```python
from build123d import *

# Parameters (mm, degrees)
FILLET_1_R                           = 18
FILLET_2_R                           = 4
SKETCH_2_R                           = 13
CUT_EXTRUDE_1_DEPTH                  = 440.177071421
CHAMFER_1_SIZE                       = 2
PATTERN_CIRCULAR_1_COUNT             = 10
CHAMFER_1_OF_PATTERN_CIRCULAR_1_SIZE = 2


with BuildPart() as part:
    # 草图1 → 旋转1 (revolve)
    with BuildSketch(Plane.XY, mode=Mode.PRIVATE) as revolve_1_sk:
        Polygon((0, 309.5), (36, 309.5), (36, 140.5), (24, 140.5), (24, 217.5), (22, 217.5), (22, 295.5), (0, 295.5), align=None)
    revolve(revolve_1_sk.sketch.rotate(Axis((-295.4, 0, 0), (1, 0, 0)), 90), axis=Axis((-295.4, 0, 0), (1, 0, 0)))

    # 圆角1
    fillet_1_edges = [part.edges().sort_by_distance(p)[0] for p in [
        (36, 0, -309.5),
    ]]
    fillet(fillet_1_edges, radius=FILLET_1_R)

    # 圆角2
    fillet_2_edges = [part.edges().sort_by_distance(p)[0] for p in [
        (22, 0, -295.5),
    ]]
    fillet(fillet_2_edges, radius=FILLET_2_R)

    # 草图2 → 切除-拉伸1 (cut, through all)
    with BuildSketch(Plane(origin=(36, 0, 0), x_dir=(0, 0, -1), z_dir=(1, 0, 0))):
        with Locations((0, 167.5)):
            Circle(SKETCH_2_R)
    cut_extrude_1 = extrude(amount=-CUT_EXTRUDE_1_DEPTH, mode=Mode.SUBTRACT)

    # 倒角1
    chamfer_1_edges = [part.edges().sort_by_distance(p)[0] for p in [
        (24, 167.5, 13),
    ]]
    chamfer(chamfer_1_edges, length=CHAMFER_1_SIZE)

    # 草图3 → 切除-旋转1 (revolve, cut)
    with BuildSketch(Plane.XY, mode=Mode.PRIVATE) as cut_revolve_1_sk:
        with BuildLine():
            Line((32.398120874, 180.50807098), (32.398120874, 167.5))
            Line((32.398120874, 167.5), (65.246950766, 167.5))
            ThreePointArc((65.246950766, 167.5), (53.242386137, 185.165329999), (32.398120874, 180.50807098))
        make_face()
    cut_revolve_1 = revolve(cut_revolve_1_sk.sketch.rotate(Axis((0, 167.5, 0), (1, 0, 0)), 270), axis=Axis((0, 167.5, 0), (1, 0, 0)), mode=Mode.SUBTRACT)

    # 阵列(圆周)1: 切除-拉伸1, 切除-旋转1 ×10 about axis
    pattern_circular_1_axis = Axis((0, 0, 0), (1, 0, 0))
    add([cut_extrude_1.rotate(pattern_circular_1_axis, i * 360 / PATTERN_CIRCULAR_1_COUNT) for i in range(1, PATTERN_CIRCULAR_1_COUNT)], mode=Mode.SUBTRACT)
    add([cut_revolve_1.rotate(pattern_circular_1_axis, i * 360 / PATTERN_CIRCULAR_1_COUNT) for i in range(1, PATTERN_CIRCULAR_1_COUNT)], mode=Mode.SUBTRACT)

    # 倒角1 of 阵列(圆周)1
    chamfer_1_of_pattern_circular_1_edges = [part.edges().sort_by_distance(p)[0] for p in [
        (24, 127.869138278, 108.971250686),
        (24, 39.396611846, 163.319187406),
        (24, -64.12408127, 155.284745553),
        (24, -143.151554838, 87.936808832),
        (24, -167.5, -13),
        (24, -127.869138278, -108.971250686),
        (24, -39.396611846, -163.319187406),
        (24, 64.12408127, -155.284745553),
        (24, 143.151554838, -87.936808832),
    ]]
    chamfer(chamfer_1_of_pattern_circular_1_edges, length=CHAMFER_1_OF_PATTERN_CIRCULAR_1_SIZE)


solid = part.part
```
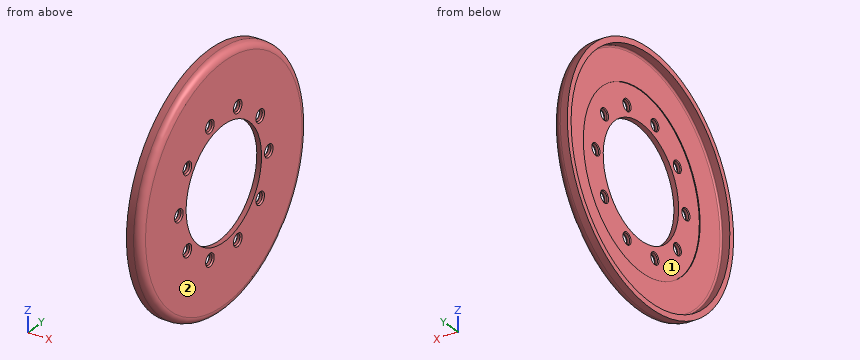
Work out the finished part from the listing and answer in its coordinate system (mm). Face numbers are marked on the shaded views. A direction names the side the tool comes from. Give positions to 0.01 mm unless a question says otherwise; leave off trailing zeros. Loops run counter-clockwise (first coordinate to the right, second up) from the corner with the lowest first, then second, coordinate; pieces in that order, holes last. Notation, with made-up numbers: (39, -1.75) - (83, -1.75) arc R15 ccw to (83, 26.25) - close; hole circle Ø8 at (81, -16.5). An arc over 180 degrees is marked (long way). Use CSV: the item, a comma, the result in double quotes. Start each with the question number.
(1) Each of these flat-tipped pins is pushed along its axis until it touches: pin 1 (12 mm diameter, centred on x = 15, z = 90.5, fed in from +Y); pin 2 (10 mm diameter, centred on x = 5.5, y = -123.5, fed in from +Z); pin 3 (1.5 mm diameter, centred on x = 11.5, y = 239, fed in from +Z); pin 4 (21 mm diameter, centred on y = 51.76, z = 159.3, fed in from -X). Where does it stop, or does it pass through?
(2) Find the intervals of material crossed by L1, parallel to X at y = -75, z = 252; L2, parallel to X at y = 28, z = 213; L3, parallel to Y at x = 5, z = -140, in increasing order.
(3) Find section C-C, the plane x = 6. Determine the outline of the cut face in (y, z).
(4) A tool of negligible diameter and unlimited length cuts with its end or side. For the marked faces 1 and 2, from which of +Z, -Z, +X, -X, +Y, -Y can it reach the whole face along a straight path? Write none if from no direction.
(5) Find section B-B, the plane z = 0. Count the separate pieces of the cut face and the enclosed holes in it, plus the area to 3 significant figures.
(6) Find section A-A, the plane y = 0. Determine the outline of the cut face in (x, z), plus the area to 3 significant figures.
Results found:
1,pin 1,"y = 297.74"
1,pin 2,"z = 285.92"
1,pin 3,"z = 197.55"
1,pin 4,"through"
2,L1,"22 to 36"
2,L2,"24 to 36"
2,L3,"-276.03 to -260.23, 260.23 to 276.03"
3,outline,"circle Ø619 at (0, 0); hole circle Ø591 at (0, 0)"
4,face 1,"-X"
4,face 2,"+Z, -Z, +X, +Y, -Y"
5,separate pieces,"4"
5,enclosed holes,"0"
5,area,"4,250 mm^2"
6,outline,"(0, -309.5) - (18, -309.5) arc R18 ccw to (36, -291.5) - (36, -140.5) - (24, -140.5) - (24, -217.5) - (22, -217.5) - (22, -291.5) arc R4 cw to (18, -295.5) - (0, -295.5) - close; (0, 295.5) - (18, 295.5) arc R4 cw to (22, 291.5) - (22, 217.5) - (24, 217.5) - (24, 140.5) - (36, 140.5) - (36, 291.5) arc R18 ccw to (18, 309.5) - (0, 309.5) - close"
6,area,"4,910 mm^2"
